from build123d import *

# Parameters (mm, degrees)
SKETCH1_W                = 380
SKETCH1_H                = 80
BOSS_EXTRUDE1_DEPTH      = 18
F_1_1_4_7_TAPPED_HOLE1_D = 28.17876


with BuildPart() as part:
    # Sketch1 → Boss-Extrude1 (new, symmetric)
    with BuildSketch(Plane.XY):
        Rectangle(SKETCH1_W, SKETCH1_H)
    extrude(amount=BOSS_EXTRUDE1_DEPTH, both=True)

    # 1-1/4-7 Tapped Hole1 (through all)
    with Locations(Plane.XY.offset(18)):
        with Locations((-150, 0), (150, 0)):
            Hole(F_1_1_4_7_TAPPED_HOLE1_D / 2)


solid = part.part
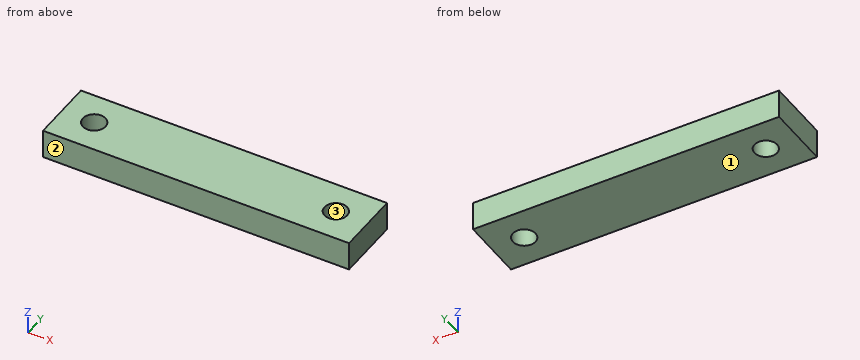
Design review of the part built by this model. Coordinates are the model's own, in mm. Face numbers are marked on the shaded views. Coordinates: 2 decimals unless noted, no trailing zeros. Order: outer loops, then holes, each group sorted by start corner. A loop starts at its lowest first (then second) coordinate and runs counter-clockwise, first axis right, second up.
Item 1: For line 1 (Y direction, x = 150, z = -7); line 2 (X direction, y = -1, z = 13.5); line 3 (X direction, y = -5, z = 11.5), list the stretches that pass through material, from the lowest coordinate up.
Item 2: Take a section at A-A, the plane x = -150. Write out the cut boundary in (y, z).
Item 3: The part is to be moulded in two halves that separate along Y. For the marked faces 1, 2 and 3, say which applies: pulls with the +Y half, pulls with the -Y half, needs draft (parallel to the pull), parting line crosses it, or undercut.
Item 4: Take a section at C-C, the plane z = -12. Write out the cut boundary in (x, y).
Item 5: Take a section at B-B, the plane y = 0. Write out the cut boundary in (x, z), then the cut area to 3 significant figures.
The answers:
1. line 1: y = -40 to -14.09, 14.09 to 40
1. line 2: x = -190 to -164.05, -135.95 to 135.95, 164.05 to 190
1. line 3: x = -190 to -163.17, -136.83 to 136.83, 163.17 to 190
2. outline: (-40, -18) - (-14.09, -18) - (-14.09, 18) - (-40, 18) - close; (14.09, -18) - (40, -18) - (40, 18) - (14.09, 18) - close
3. face 1: needs draft
3. face 2: pulls with the -Y half
3. face 3: undercut
4. outline: (-190, -40) - (190, -40) - (190, 40) - (-190, 40) - close; hole circle Ø28.18 at (-150, 0); hole circle Ø28.18 at (150, 0)
5. outline: (-190, -18) - (-164.09, -18) - (-164.09, 18) - (-190, 18) - close; (-135.91, -18) - (135.91, -18) - (135.91, 18) - (-135.91, 18) - close; (164.09, -18) - (190, -18) - (190, 18) - (164.09, 18) - close
5. area: 11,700 mm2
